The figure shows three views and two pictorial views of one solid part (mm, origin at its lowest corner). Answer the questions. A direction names the side the tool comes from. Give positions to 0.01 mm unless a question says otherwise; leave off trailing zeros. Loops run counter-clockwise (first coordinate to the right, second up) from the corner with the lowest first, then second, coordinate; pieces in that order, holes last.
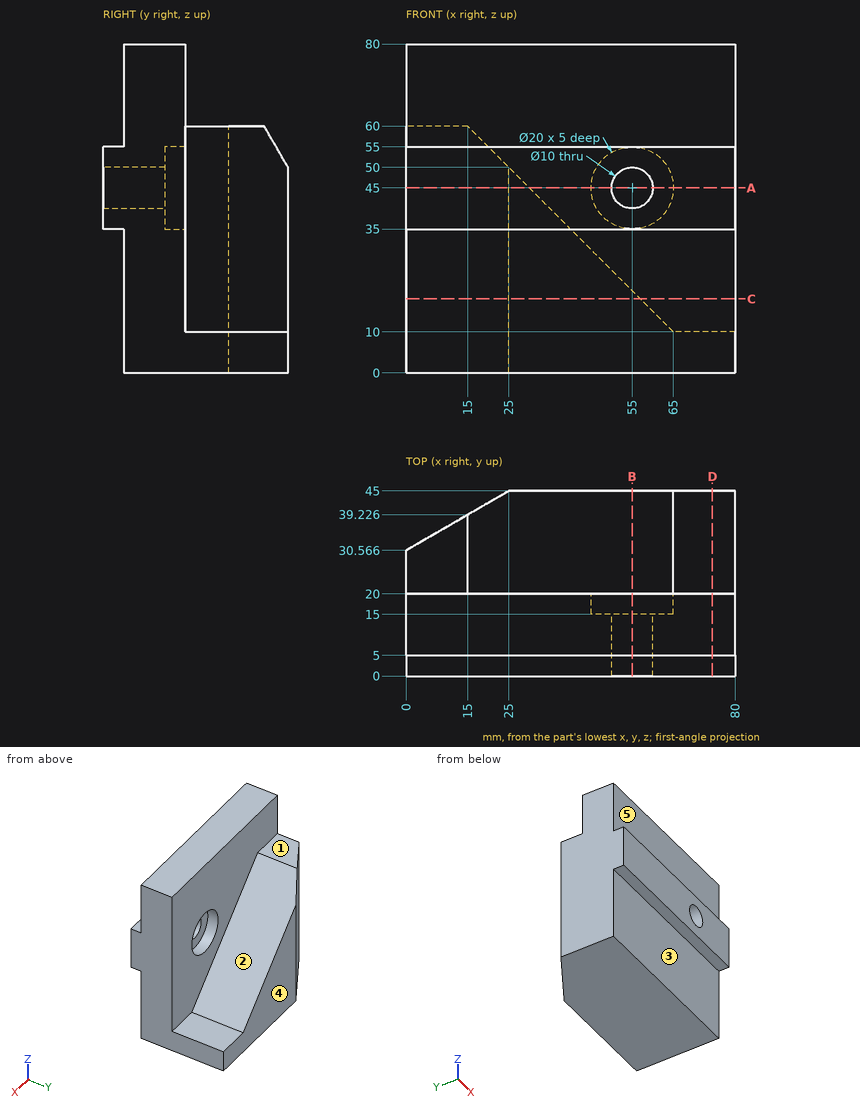
Q1. Consider line 1 along X through (y, z) = (5.75, 45); line 2 along Z through (x, y) = (75, 26.5); line 3 along Y through (x, z) = (74, 50.5). Determine where each line is inside the solid, lowest interval first.
Q2. Section A-A on z = 45 is taken. Give the vertices of the cut face in (x, y), plus the area to 3 significant figures.
Q3. Section D-D on x = 74.5 is taken. Give the vertices of the cut face in (y, z).
Q4. Given pin 1 (4 mm diameter, centred on x = 35, z = 43.5, fed in from -Y); pin 2 (7.5 mm diameter, centred on x = 71.5, y = 33, fed in from +Z); pin 3 (2.5 mm diameter, centred on x = 31, y = 2.5, fed in from +Z); pin 4 (6 mm diameter, centred on x = 55, z = 45, fed in from +Y), each flat-ended and moving along its own axis, determine where each tip first touches the part or whether it passes through.
Q5. Section B-B on x = 55 is taken. Give the vertices of the cut face in (y, z), plus the area to 3 significant figures.
Q6. Which of the six approach directions +Z, -Z, +X, -X, +Y, -Y give full straight-line access (tool end or side, diameter ignored) to the marked faces 1, 2, 3, 4 and 5?
Q7. Section C-C on z = 18 is taken. Give the vertices of the cut face in (x, y), plus the area to 3 significant figures.
Check result:
1. line 1: x = 0 to 50, 60 to 80
1. line 2: z = 0 to 10
1. line 3: y = 0 to 20
2. outline: (0, 0) - (50, 0) - (50, 15) - (45, 15) - (45, 20) - (30, 20) - (30, 45) - (25, 45) - (0, 30.57) - close; (60, 0) - (80, 0) - (80, 20) - (65, 20) - (65, 15) - (60, 15) - close
2. area: 1,920 mm2
3. outline: (0, 35) - (5, 35) - (5, 0) - (45, 0) - (45, 10) - (20, 10) - (20, 80) - (5, 80) - (5, 55) - (0, 55) - close
4. pin 1: stops at y = 0
4. pin 2: stops at z = 10
4. pin 3: stops at z = 55
4. pin 4: passes through
5. outline: (0, 35) - (5, 35) - (5, 0) - (45, 0) - (45, 20) - (20, 20) - (20, 35) - (15, 35) - (15, 40) - (0, 40) - close; (0, 50) - (15, 50) - (15, 55) - (20, 55) - (20, 80) - (5, 80) - (5, 55) - (0, 55) - close
5. area: 1,550 mm2
6. face 1: +Z, +X, -X, +Y
6. face 2: +Z, +X, +Y
6. face 3: -Z, +X, -X, -Y
6. face 4: +Z, -Z, +X, -X, +Y
6. face 5: +Z, +X, -X, -Y
7. outline: (0, 5) - (80, 5) - (80, 20) - (57, 20) - (57, 45) - (25, 45) - (0, 30.57) - close
7. area: 2,440 mm2
